```python
from build123d import *

# Parameters (mm, degrees)
BOSS_EXTRUDE1_DEPTH = 1.6


with BuildPart() as part:
    # Sketch1 → Boss-Extrude1 (new, symmetric)
    with BuildSketch(Plane.XY):
        Polygon((30.5, 25), (50.3, 25), (50.3, 30), (53.3, 30), (53.3, 45), (50.3, 45), (50.3, 50), (30.5, 50), (30.5, 45), (27.5, 45), (27.5, 30), (30.5, 30), align=None)
    extrude(amount=BOSS_EXTRUDE1_DEPTH, both=True)


solid = part.part
```
Build history of the part. All positions in model axes, mm. A direction names the side the tool comes from. Give positions to 0.01 mm unless a question says otherwise; leave off trailing zeros. Order: outer loops, then holes, each group sorted by start corner. A loop starts at its lowest first (then second) coordinate and runs counter-clockwise, first axis right, second up. Notation, with made-up numbers: M -9,-10.75 L 46,-10.75 A18 ccw 46,-3.75 Z; hole C 29,70 d6. An arc over 180 degrees is marked long. Return JSON: item names as keys, results as strings.
Q1. Flat gauge pins, fed straight in: pin 1 (1 mm diameter, centred on y = 46.5, z = 0.5, fed in from +X); pin 2 (1.5 mm diameter, centred on x = 29, z = 0, fed in from +Y); pin 3 (1.6 mm diameter, centred on y = 26.5, z = 0, fed in from -X). Where does each tip first touch, or does it go through?
Answer list:
{"pin 1": "stops at x = 50.3", "pin 2": "stops at y = 45", "pin 3": "stops at x = 30.5"}
Q2. Band-saw the part on B-B (y = 48.25). Give the cut face in (x, z), then the cut area to 3 significant figures.
Answer list:
{"outline": "M 30.5,-1.6 L 50.3,-1.6 L 50.3,1.6 L 30.5,1.6 Z", "area": "63.4 mm^2"}
Q3. 3-axis set-ups, long thin cutter, end or side, ignore diameter. For faces 1 (the face through (30.5, 28, 0)), 2 (the face through (50.3, 27, 0)), 3 (the face through (30.5, 48, 0)): which of +Z, -Z, +X, -X, +Y, -Y reach the whole face in a straight line?
Answer list:
{"face 1": "+Z, -Z, -X, -Y", "face 2": "+Z, -Z, +X, -Y", "face 3": "+Z, -Z, -X, +Y"}
Q4. Band-saw the part on A-A (z = -0.2). Give the cut face in (x, y).
Answer list:
{"outline": "M 27.5,30 L 30.5,30 L 30.5,25 L 50.3,25 L 50.3,30 L 53.3,30 L 53.3,45 L 50.3,45 L 50.3,50 L 30.5,50 L 30.5,45 L 27.5,45 Z"}
Q5. Wall check: probe 1 along X at (y, z) = (48.5, -0.8); probe 2 along Y at (x, z) = (29.5, -0.3). Give the ranges that are in metal, low to high. Write a range as from..to.
Answer list:
{"probe 1": "x = 30.5..50.3", "probe 2": "y = 30..45"}
